from build123d import *

# Parameters (mm, degrees)
SKETCH1_W            = 360
SKETCH1_H            = 320
EXTRUDE1_DEPTH       = 8
EXTRUDE2_DEPTH       = 16
SKETCH3_R            = 8.5
EXTRUDE3_DEPTH       = 16
LPATTERN1_COUNT      = 2
LPATTERN1_PITCH      = 240
LPATTERN1_COUNT_DIR2 = 2
LPATTERN1_PITCH_DIR2 = 168


with BuildPart() as part:
    # Sketch1 → Extrude1 (new, symmetric)
    with BuildSketch(Plane.XY):
        Rectangle(SKETCH1_W, SKETCH1_H)
    extrude(amount=EXTRUDE1_DEPTH, both=True)

    # Sketch2 → Extrude2 (cut)
    with BuildSketch(Plane.XY.offset(8)):
        with BuildLine():
            Line((-60, -160), (-60, -30))
            ThreePointArc((-60, -30), (0, 30), (60, -30))
            Line((60, -30), (60, -160))
            Line((60, -160), (-60, -160))
        make_face()
    extrude(amount=-EXTRUDE2_DEPTH, mode=Mode.SUBTRACT)

    # Sketch3 → Extrude3 (cut)
    with BuildSketch(Plane.XY.offset(8)):
        with Locations((-120, 63)):
            Circle(SKETCH3_R)
    extrude3 = extrude(amount=-EXTRUDE3_DEPTH, mode=Mode.SUBTRACT)

    # LPattern1: Extrude3 2 × 2
    with Locations(*[(i * LPATTERN1_PITCH, -j * LPATTERN1_PITCH_DIR2, 0) for i in range(LPATTERN1_COUNT) for j in range(LPATTERN1_COUNT_DIR2) if (i, j) != (0, 0)]):
        add(extrude3, mode=Mode.SUBTRACT)


solid = part.part
Geometry: final body of the model. Coordinates: model frame, mm. A direction names the side the tool comes from. Coordinates: 2 decimals unless noted, no trailing zeros. Order: outer loops, then holes, each group sorted by start corner. A loop starts at its lowest first (then second) coordinate and runs counter-clockwise, first axis right, second up.
1) Set-up query: faces 5 (the cylindrical face through (127.85, 59.74, 0.11)), 6 (the flat face through (-60, -96, 0)). Return all of +Z, -Z, +X, -X, +Y, -Y with unobstructed straight access to the full face (end or side cutting, diameter ignored); none if empty.
Result sheet:
face 5: +Z, -Z
face 6: +Z, -Z, -Y
2) Section D-D (z = -2.5). Return loops of the section in (x, y).
Result sheet:
outline: (-180, -160) - (-60, -160) - (-60, -30) arc R60 cw to (60, -30) - (60, -160) - (180, -160) - (180, 160) - (-180, 160) - close; hole circle Ø17 at (-120, -105); hole circle Ø17 at (-120, 63); hole circle Ø17 at (120, -105); hole circle Ø17 at (120, 63)
3) Section C-C (y = -105). Return loops of the section in (x, z).
Result sheet:
outline: (-180, -8) - (-128.5, -8) - (-128.5, 8) - (-180, 8) - close; (-111.5, -8) - (-60, -8) - (-60, 8) - (-111.5, 8) - close; (60, -8) - (111.5, -8) - (111.5, 8) - (60, 8) - close; (128.5, -8) - (180, -8) - (180, 8) - (128.5, 8) - close
4) Ray query, probe 1 along Y at (x, z) = (120, -3); probe 2 along Y at (x, z) = (-119, 4.75); probe 3 along X at (y, z) = (-64, 4.75). Return the intervals inside material, ascending.
Result sheet:
probe 1: y = -160 to -113.5, -96.5 to 54.5, 71.5 to 160
probe 2: y = -160 to -113.44, -96.56 to 54.56, 71.44 to 160
probe 3: x = -180 to -60, 60 to 180
5) Section A-A (y = 63). Return loops of the section in (x, z).
Result sheet:
outline: (-180, -8) - (-128.5, -8) - (-128.5, 8) - (-180, 8) - close; (-111.5, -8) - (111.5, -8) - (111.5, 8) - (-111.5, 8) - close; (128.5, -8) - (180, -8) - (180, 8) - (128.5, 8) - close
6) Draft query along Y for faces 1 (the cylindrical face through (-1.319, 29.985, 0.112)), 2 (the cylindrical face through (-112.15, 59.74, 0.11)), 3 (the flat face through (180, -2, 0)), 4 (the cylindrical face through (123.92, -112.54, 0.11)). Return one class per face: released by +Y, released by -Y, zero draft, split by the parting line, or undercut.
Result sheet:
face 1: released by -Y
face 2: undercut
face 3: zero draft
face 4: undercut
7) Section B-B (x = 120). Return loops of the section in (y, z), then the cut area to 3 significant figures.
Result sheet:
outline: (-160, -8) - (-113.5, -8) - (-113.5, 8) - (-160, 8) - close; (-96.5, -8) - (54.5, -8) - (54.5, 8) - (-96.5, 8) - close; (71.5, -8) - (160, -8) - (160, 8) - (71.5, 8) - close
area: 4,580 mm2
